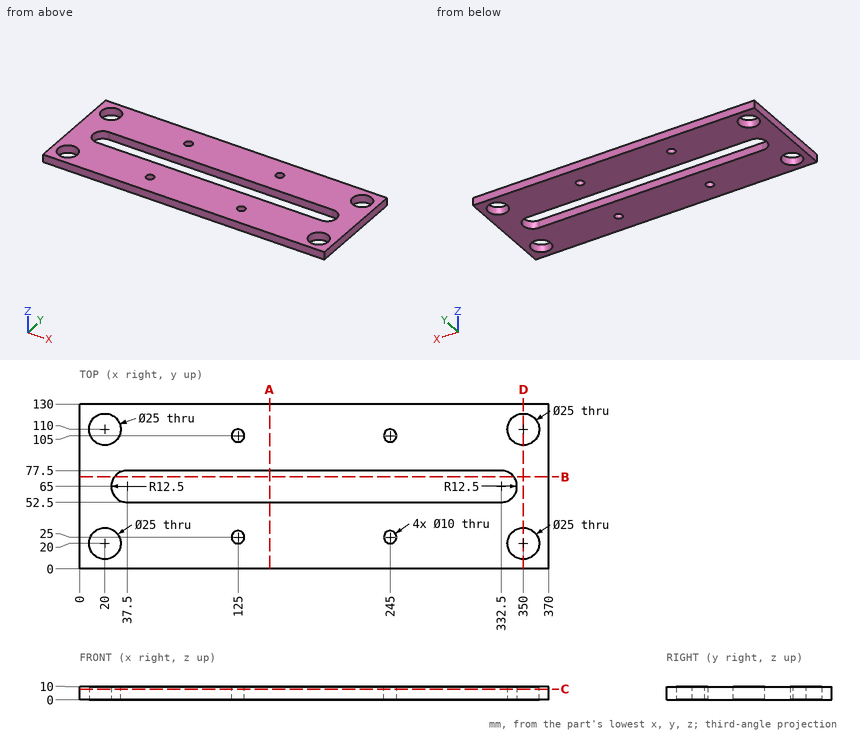
For this review, use the dimensioned drawing (mm, ordinates from the lowest corner) and the shaded views. Give positions to 0.01 mm unless a question says otherwise; leave off trailing zeros. Loops run counter-clockwise (first coordinate to the right, second up) from the corner with the lowest first, then second, coordinate; pieces in that order, holes last.
Item 1: Take a section at A-A, the plane x = 150. State the section outline as (y, z) points, and give its area (3 significant figures).
Item 2: Take a section at B-B, the plane y = 72.5. State the section outline as (x, z) points, and give its area (3 significant figures).
Item 3: Take a section at D-D, the plane x = 350. State the section outline as (y, z) points, and give its area (3 significant figures).
Item 4: Take a section at C-C, the plane z = 8.25. Give the number of separate pieces and of enclosed holes in the cut face, and give its area (3 significant figures).
Item 5: Insertion check: pin 1 (15 mm diameter, centred on x = 350, y = 110, fed in from -Z). The pin has a flat end and moves straight along its axis. Give the tip position at first contact, or say it passes through.
Item 6: For line 1 along Y through (x, z) = (245, 5.5); line 2 along X through (y, z) = (109.5, 1.25); line 3 along Y through (x, z) = (143, 1.25), list the stretches that pass through material, from the lowest coordinate up.
Calculated:
1. outline: (0, 0) - (52.5, 0) - (52.5, 10) - (0, 10) - close; (77.5, 0) - (130, 0) - (130, 10) - (77.5, 10) - close
1. area: 1,050 mm2
2. outline: (0, 0) - (27.5, 0) - (27.5, 10) - (0, 10) - close; (342.5, 0) - (370, 0) - (370, 10) - (342.5, 10) - close
2. area: 550 mm2
3. outline: (0, 0) - (7.5, 0) - (7.5, 10) - (0, 10) - close; (32.5, 0) - (97.5, 0) - (97.5, 10) - (32.5, 10) - close; (122.5, 0) - (130, 0) - (130, 10) - (122.5, 10) - close
3. area: 800 mm2
4. separate pieces: 1
4. enclosed holes: 9
4. area: 38,000 mm2
5. pin 1: passes through
6. line 1: y = 0 to 20, 30 to 52.5, 77.5 to 100, 110 to 130
6. line 2: x = 0 to 7.51, 32.49 to 122.82, 127.18 to 242.82, 247.18 to 337.51, 362.49 to 370
6. line 3: y = 0 to 52.5, 77.5 to 130
